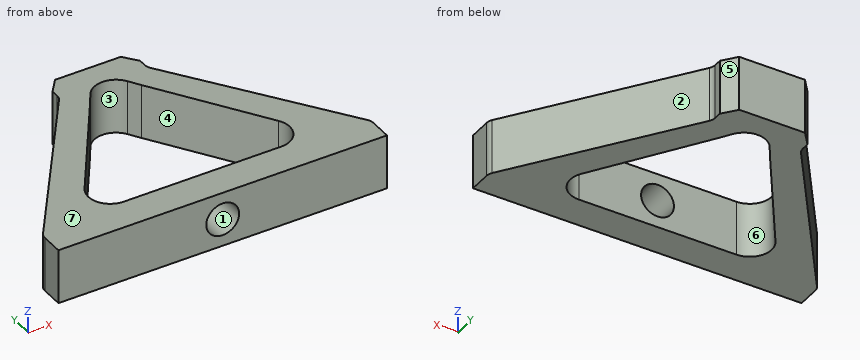
from build123d import *

# Parameters (mm, degrees)
EXTRUDE_1_DEPTH     = 10
SKETCH_3_R          = 3
CUT_EXTRUDE_1_DEPTH = 10


with BuildPart() as part:
    # 草图1 → 凸台-拉伸1 (new body)
    with BuildSketch(Plane.XY):
        with BuildLine():
            Line((-36.484728771, -19.952952756), (23.515271229, -19.952952756))
            Line((23.515271229, -19.952952756), (23.515271229, -15.952952756))
            ThreePointArc((23.515271229, -15.952952756), (23.429409838, -15.373234389), (23.179197844, -14.843291448))
            Line((23.179197844, -14.843291448), (1.886808682, 15.02014861))
            ThreePointArc((1.886808682, 15.02014861), (1.61041886, 15.571691167), (1.515271229, 16.181229888))
            Line((1.515271229, 16.181229888), (1.515271229, 17.541244626))
            Line((1.515271229, 17.541244626), (-0.484728771, 20.047047244))
            Line((-0.484728771, 20.047047244), (-12.484728771, 20.047047244))
            Line((-12.484728771, 20.047047244), (-14.484728771, 17.541244626))
            Line((-14.484728771, 17.541244626), (-14.484728771, 16.181229888))
            ThreePointArc((-14.484728771, 16.181229888), (-14.579876402, 15.571691167), (-14.856266224, 15.02014861))
            Line((-14.856266224, 15.02014861), (-36.148451723, -14.842986118))
            ThreePointArc((-36.148451723, -14.842986118), (-36.39881418, -15.373058759), (-36.484728771, -15.952952756))
            Line((-36.484728771, -15.952952756), (-36.484728771, -19.952952756))
        make_face()
        with BuildLine():
            Line((-24.192238855, -7.733019479), (-11.181735098, 11.768353778))
            Line((-11.181735098, 11.768353778), (-9.853193624, 13.848209774))
            ThreePointArc((-9.853193624, 13.848209774), (-6.483571586, 15.694946417), (-3.112703027, 13.850486044))
            Line((-3.112703027, 13.850486044), (-1.802931634, 11.803064426))
            Line((-1.802931634, 11.803064426), (11.2259567, -7.733630139))
            ThreePointArc((11.2259567, -7.733630139), (11.424949828, -11.840107961), (7.89810347, -13.952952756))
            Line((7.89810347, -13.952952756), (-20.864792951, -13.952952756))
            ThreePointArc((-20.864792951, -13.952952756), (-24.391812451, -11.839784346), (-24.192238855, -7.733019479))
        make_face(mode=Mode.SUBTRACT)
    extrude(amount=EXTRUDE_1_DEPTH)

    # 草图3 → 切除-拉伸1 (cut)
    with BuildSketch(Plane.XZ.offset(19.952952756)):
        with Locations((-6.484728771, 5)):
            Circle(SKETCH_3_R)
    extrude(amount=-CUT_EXTRUDE_1_DEPTH, mode=Mode.SUBTRACT)


solid = part.part
Can you work these out from the model? Positions are in its coordinate system, mm. Face numbers are marked on the shaded views. A direction names the side the tool comes from. Round coordinates to 2 decimals unless told otherwise and drop trailing zeros. Order: outer loops, then holes, each group sorted by start corner. A loop starts at its lowest first (then second) coordinate and runs counter-clockwise, first axis right, second up. Notation, with made-up numbers: (2, 5) - (36, 5) arc R28 cw to (36, 42) - close; hole circle Ø6 at (46.5, 57.25). An arc over 180 degrees is marked (long way). Answer in a Markdown table with one row per item.
(1) Suppose I cut it at A-A, the plane z = 5. Please give me the cut outline in (x, y), plus the area to 3 significant figures.
From the geometry:
| item | result |
|---|---|
| outline | (-36.48, -19.95) - (-9.48, -19.95) - (-9.48, -13.95) - (-20.86, -13.95) arc R4 cw to (-24.19, -7.73) - (-11.18, 11.77) - (-9.85, 13.85) arc R4 cw to (-3.11, 13.85) - (-1.8, 11.8) - (11.23, -7.73) arc R4 cw to (7.9, -13.95) - (-3.48, -13.95) - (-3.48, -19.95) - (23.52, -19.95) - (23.52, -15.95) arc R2 ccw to (23.18, -14.84) - (1.89, 15.02) arc R2 cw to (1.52, 16.18) - (1.52, 17.54) - (-0.48, 20.05) - (-12.48, 20.05) - (-14.48, 17.54) - (-14.48, 16.18) arc R2 cw to (-14.86, 15.02) - (-36.15, -14.84) arc R2 ccw to (-36.48, -15.95) - close |
| area | 798 mm2 |
(2) Which directions (+Z, -Z, +X, -X, +Y, -Y) give clear straight access to the entire face, cutting with the end or side of a thin tool? Please do the marked faces 1, 2 and 3.
From the geometry:
| item | result |
|---|---|
| face 1 | -Y |
| face 2 | +Z, -Z, +X, +Y |
| face 3 | +Z, -Z |
(3) If we mould it in two halves opening along X, with no side actions, what happens to the marked faces 4, 5, 6 and 7? For each: released by +X, released by -X, zero draft, split by the parting line, or undercut.
From the geometry:
| item | result |
|---|---|
| face 4 | undercut |
| face 5 | released by +X |
| face 6 | undercut |
| face 7 | zero draft |
(4) For P1, Ø1.5, axis at y = 2, z = 6, coming from the -X side; P2, Ø1, axis at y = -8, z = 2, coming from the +X side; P3, Ø2, axis at y = 10, z = 4.5, coming from the +X side, each with a flat end and sliding along its axis, tell me the tip position at first contact or that it passes through.
From the geometry:
| item | result |
|---|---|
| P1 | stops at x = -24.67 |
| P2 | stops at x = 18.66 |
| P3 | stops at x = 6.18 |
(5) Suppose I cut it at C-C, the plane x = -6. Please give me the cut outline in (y, z).
From the geometry:
| item | result |
|---|---|
| outline | (-19.95, 0) - (-13.95, 0) - (-13.95, 2.04) - (-19.95, 2.04) - close; (-19.95, 7.96) - (-13.95, 7.96) - (-13.95, 10) - (-19.95, 10) - close; (15.67, 0) - (20.05, 0) - (20.05, 10) - (15.67, 10) - close |
(6) Please list where these lines run through material, in increasing order: L1, parallel to X at y = 15, z = 9.5; L2, parallel to Y at x = 0.5, z = 8.5; L3, parallel to Y at x = -9.5, z = 6.75. Write a range as from..to.
From the geometry:
| item | result |
|---|---|
| L1 | x = -14.87..-8.74, -4.23..1.9 |
| L2 | y = -19.95..-13.95, 8.35..18.81 |
| L3 | y = -19.95..-13.95, 14.32..20.05 |
(7) Suppose I cut it at B-B, the plane x = 2.5. Please give me the cut outline in (y, z), plus the area to 3 significant figures.
From the geometry:
| item | result |
|---|---|
| outline | (-19.95, 0) - (-13.95, 0) - (-13.95, 10) - (-19.95, 10) - close; (5.35, 0) - (14.16, 0) - (14.16, 10) - (5.35, 10) - close |
| area | 148 mm2 |
